Input: part model. Units: mm. Frame: model coordinates. A direction names the side the tool comes from. Give positions to 0.01 mm unless a question says otherwise; leave off trailing zeros. Write each loop counter-clockwise with the first axis right and the second up, starting at its lowest first coordinate (ties: lowest second). Pieces come first, ordered by that corner, then holes.
```python
from build123d import *

# Parameters (mm, degrees)
SKETCH_1_W                   = 70
SKETCH_1_H                   = 72.5
EXTRUDE_1_DEPTH              = 10
SKETCH_2_W                   = 2
SKETCH_2_H                   = 10
CUT_EXTRUDE_1_DEPTH          = 80.461075377
HOLE_WIZARD_M5_1_D           = 5.5
HOLE_WIZARD_M5_1_CBORE_D     = 10
HOLE_WIZARD_M5_1_CBORE_DEPTH = 5.4
MM_1_D                       = 5
HOLE_WIZARD_M4_1_D           = 3.3
SKETCH_9_R                   = 20
CUT_EXTRUDE_2_DEPTH          = 52.37180647
CHAMFER_1_SIZE               = 5
CHAMFER_2_SIZE               = 0.5


with BuildPart() as part:
    # 草图1 → 凸台-拉伸1 (new body)
    with BuildSketch(Plane.XY):
        Rectangle(SKETCH_1_W, SKETCH_1_H)
    extrude(amount=EXTRUDE_1_DEPTH)

    # 草图2 → 切除-拉伸1 (cut, through all)
    with BuildSketch(Plane.ZY.offset(35)):
        with Locations((1, 29.25)):
            Rectangle(SKETCH_2_W, SKETCH_2_H)
    extrude(amount=-CUT_EXTRUDE_1_DEPTH, mode=Mode.SUBTRACT)

    # M5 六角凹头螺钉的柱形沉头孔1 (through all)
    with Locations(Plane.XY.offset(10)):
        with Locations((27.5, 29.25), (-27.5, 29.25)):
            CounterBoreHole(HOLE_WIZARD_M5_1_D / 2, HOLE_WIZARD_M5_1_CBORE_D / 2, HOLE_WIZARD_M5_1_CBORE_DEPTH)

    # 大小mm 暗销孔1 (through all)
    with Locations(Plane.XY.offset(10)):
        with Locations((0, 29.25)):
            Hole(MM_1_D / 2)

    # M4 螺纹孔1 (through all)
    with Locations(Plane.XY.offset(10)):
        with Locations((-23.57, 15.82), (-23.57, -31.32), (23.57, -31.32), (23.57, 15.82)):
            Hole(HOLE_WIZARD_M4_1_D / 2)

    # 草图9 → 切除-拉伸2 (cut, through all)
    with BuildSketch(Plane(origin=(0, 0, 0), x_dir=(-1, 0, 0), z_dir=(0, 0, -1))):
        with Locations((0, -7.75)):
            Circle(SKETCH_9_R)
    extrude(amount=-CUT_EXTRUDE_2_DEPTH, mode=Mode.SUBTRACT)

    # 倒角1
    chamfer_1_edges = [part.edges().sort_by_distance(p)[0] for p in [
        (35, -36.25, 5),
        (-35, -36.25, 5),
    ]]
    chamfer(chamfer_1_edges, length=CHAMFER_1_SIZE)

    # 倒角2
    chamfer_2_edges = [part.edges().sort_by_distance(p)[0] for p in [
        (35, 2.5, 10),
        (35, -3.5, 0),
        (0, -36.25, 0),
        (-32.5, -33.75, 0),
        (32.5, -33.75, 0),
        (0, -36.25, 10),
        (-32.5, -33.75, 10),
        (32.5, -33.75, 10),
        (-35, 2.5, 10),
        (35, 35.25, 0),
        (-35, -3.5, 0),
        (-35, 35.25, 0),
        (0, 36.25, 0),
        (-35, 36.25, 5),
        (35, 36.25, 5),
        (0, 36.25, 10),
    ]]
    chamfer(chamfer_2_edges, length=CHAMFER_2_SIZE)


solid = part.part
```
Q1. Mould query, pull axis Y, two halves, no side actions, for faces 1 (the flat face through (0, 36.25, 5)), 2 (the cylindrical face through (0.33, 31.73, 5.94)), 3 (the flat face through (32.29, -33.61, 9.75)). Classes: +Y half, -Y half, draft (parallel to the pull), parting line (faces both ways), or undercut.
Q2. Section C-C, the plane z = 3.25. Give the number of separate pieces and of enclosed holes in the cut face, then the cut area to 3 significant figures.
Q3. Material intervals for line 1 along Y through (x, z) = (23.57, 4.5); line 2 along X through (y, z) = (-8, 3.5); line 3 along Y through (x, z) = (-27.5, 4), sorted ascending.
Q4. Section A-A, the plane y = -7.75. Return the cut outline in (x, z).
Q5. Section D-D, the plane y = 15.82. Return the cut outline in (x, z).
Q6. Pin query (flat end, axial travel): pin 1 (9 mm diameter, centred on x = 27.5, y = 29.25, fed in from +Z); pin 2 (4 mm diameter, centred on x = 23.57, y = 15.82, fed in from -Z); pin 3 (8 mm diameter, centred on x = -7.5, y = 28.5, fed in from -Z). Return the tip coordinate at first contact, or that it passes through.
Q7. Access query for faces 4 (the cylindrical face through (21.996, 16.316, 4.93)), 5 (the flat face through (30, 27, 4.6)), 6 (the flat face through (0, 34.25, 1)). Directions: +Z, -Z, +X, -X, +Y, -Y. A direction counts if a zero-diameter tool reaches every point of the face in a straight line with its end or side. Return the directions, or none.
Q8. Section B-B, the plane x = 0. Return the cut outline in (y, z).
Solutions:
1. face 1: +Y half
1. face 2: undercut
1. face 3: -Y half
2. separate pieces: 1
2. enclosed holes: 8
2. area: 3,690 mm2
3. line 1: y = -36.25 to -32.97, -29.67 to 14.17, 17.47 to 36.25
3. line 2: x = -35 to -20, 20 to 35
3. line 3: y = -36.25 to 26.5, 32 to 36.25
4. outline: (-35, 0.5) - (-34.5, 0) - (-20, 0) - (-20, 10) - (-34.5, 10) - (-35, 9.5) - close; (20, 0) - (34.5, 0) - (35, 0.5) - (35, 9.5) - (34.5, 10) - (20, 10) - close
5. outline: (-35, 0.5) - (-34.5, 0) - (-25.22, 0) - (-25.22, 10) - (-34.5, 10) - (-35, 9.5) - close; (-21.92, 0) - (21.92, 0) - (21.92, 10) - (-21.92, 10) - close; (25.22, 0) - (34.5, 0) - (35, 0.5) - (35, 9.5) - (34.5, 10) - (25.22, 10) - close
6. pin 1: stops at z = 4.6
6. pin 2: stops at z = 0
6. pin 3: stops at z = 2
7. face 4: +Z, -Z
7. face 5: +Z
7. face 6: -Z, +X, -X
8. outline: (-36.25, 0.5) - (-35.75, 0) - (-27.75, 0) - (-27.75, 10) - (-35.75, 10) - (-36.25, 9.5) - close; (12.25, 0) - (24.25, 0) - (24.25, 2) - (26.75, 2) - (26.75, 10) - (12.25, 10) - close; (31.75, 2) - (34.25, 2) - (34.25, 0) - (35.75, 0) - (36.25, 0.5) - (36.25, 9.5) - (35.75, 10) - (31.75, 10) - close
